```python
from build123d import *

# Parameters (mm, degrees)
SKETCH1_W           = 50
SKETCH1_H           = 50
BOSS_EXTRUDE1_DEPTH = 5
CHAMFER1_SIZE       = 5


with BuildPart() as part:
    # Sketch1 → Boss-Extrude1 (new body)
    with BuildSketch(Plane.XY):
        with Locations((0.541184779, 3.419811321)):
            Rectangle(SKETCH1_W, SKETCH1_H)
    extrude(amount=BOSS_EXTRUDE1_DEPTH)

    # Chamfer1
    chamfer1_edges = [part.edges().sort_by_distance(p)[0] for p in [
        (-24.458815221, 28.419811321, 2.5),
        (25.541184779, 28.419811321, 2.5),
        (25.541184779, -21.580188679, 2.5),
        (-24.458815221, -21.580188679, 2.5),
    ]]
    chamfer(chamfer1_edges, length=CHAMFER1_SIZE)


solid = part.part
```
The model under review builds one solid part; all positions refer to its coordinate system, in mm. Round coordinates to 2 decimals unless told otherwise and drop trailing zeros. Write each loop counter-clockwise with the first axis right and the second up, starting at its lowest first coordinate (ties: lowest second). Pieces come first, ordered by that corner, then holes. Notation, with made-up numbers: M -26.5,-25 L -11.5,-25 A16 cw -11.5,-1 Z; hole C 36.5,6.25 d6. An arc over 180 degrees is marked long. Use CSV: the item, a comma, the result in double quotes. Start each with the question number.
(1) For line 1 along Y through (x, z) = (-22, 1.85), list the stretches that pass through material, from the lowest coordinate up.
(2) We need section A-A, the plane z = 1.65. State the section outline as (x, y) points, then the cut area to 3 significant figures.
(3) Clearance check with a flat-ended pin moving along its axis: P1, Ø3, axis at x = 2, y = 10, coming from the -Z side. State where the tip first meets the part, or that it passes through.
(4) The part is to be moulded in two halves that separate along X. For faces 1 (the face through (23.076, -19.045, 2.465)), 2 (the face through (-24.459, 3, 2)), 3 (the face through (0, 4, 5)), say which applies: +X half, -X half, draft (parallel to the pull), parting line (faces both ways), or undercut.
Findings:
1,line 1,"-19.04 to 25.88"
2,outline,"M -24.46,-16.58 L -19.46,-21.58 L 20.54,-21.58 L 25.54,-16.58 L 25.54,23.42 L 20.54,28.42 L -19.46,28.42 L -24.46,23.42 Z"
2,area,"2,450 mm^2"
3,P1,"z = 0"
4,face 1,"+X half"
4,face 2,"-X half"
4,face 3,"draft"
